```python
from build123d import *

# Parameters (mm, degrees)
SKETCH1_R           = 12.5
BOSS_EXTRUDE1_DEPTH = 10
M10_TAPPED_HOLE1_D  = 8.5
CHAMFER1_SIZE       = 2


with BuildPart() as part:
    # Sketch1 → Boss-Extrude1 (new, symmetric)
    with BuildSketch(Plane.XY):
        Circle(SKETCH1_R)
    extrude(amount=BOSS_EXTRUDE1_DEPTH, both=True)

    # M10 Tapped Hole1 (through all)
    with Locations(Plane.XY.offset(10)):
        with Locations((0, 0)):
            Hole(M10_TAPPED_HOLE1_D / 2)

    # Sketch5 → Revolve1 (revolve)
    with BuildSketch(Plane(origin=(0, 0, 0), x_dir=(1, 0, 0), z_dir=(0, 1, 0))):
        Polygon((-12.5, 0), (-92.29474156, 60.272707085), (-88.678379135, 65.060391578), (-8.883637575, 4.787684494), align=None)
    revolve(axis=Axis((-12.5, 0, 0), (-0.7979474156035873, 0, -0.6027270708467937)))

    # Chamfer1
    chamfer1_edges = [part.edges().sort_by_distance(p)[0] for p in [
        (-95.911103985, 0, -55.485022591),
    ]]
    chamfer(chamfer1_edges, length=CHAMFER1_SIZE)


solid = part.part
```
Source: CAD feature listing. Evaluate the final solid. Frame: model axes, mm. A direction names the side the tool comes from. Round coordinates to 2 decimals unless told otherwise and drop trailing zeros. Loops run counter-clockwise (first coordinate to the right, second up) from the corner with the lowest first, then second, coordinate; pieces in that order, holes last.
(1) Section query A-A (x = 0). Output: boundary loops of the cut face in (y, z), and give its area (3 significant figures).
From the geometry:
outline: (-12.5, -10) - (-4.25, -10) - (-4.25, 10) - (-12.5, 10) - close; (4.25, -10) - (12.5, -10) - (12.5, 10) - (4.25, 10) - close
area: 330 mm2
(2) Section query C-C (y = -7.25). Output: boundary loops of the cut face in (x, z).
From the geometry:
outline: (-10.18, -10) - (10.18, -10) - (10.18, 10) - (-10.18, 10) - close
(3) Pull-direction query (X, two-part tool) for faces 3 (the cylindrical face through (-2.285, 3.584, -0.14)), 4 (the flat face through (0, -5, 10)), 5 (the conical face through (-94.68, -0.18, -56.91)); classes: +X half, -X half, draft (parallel to the pull), parting line (faces both ways), or undercut.
From the geometry:
face 3: undercut
face 4: draft
face 5: -X half
(4) Section query B-B (y = 0). Output: boundary loops of the cut face in (x, z).
From the geometry:
outline: (-94.71, -57.08) - (-89.88, -63.46) - (-87.08, -63.85) - (-12.5, -7.52) - (-12.5, -10) - (-4.25, -10) - (-4.25, 10) - (-12.5, 10) - (-12.5, 0) - (-16.12, 4.79) - (-94.32, -54.28) - close; (4.25, -10) - (12.5, -10) - (12.5, 10) - (4.25, 10) - close
(5) Contact query for flat-ended pins moving along their axis: pin 1 Ø4 at (x, y) = (-25.5, 0) entering from -Z; pin 2 Ø5 at (y, z) = (1.5, -48) entering from -X; pin 3 Ø2 at (y, z) = (3, -29) entering from +X. Output: stop coordinate, or through.
From the geometry:
pin 1: stops at z = -18.85
pin 2: stops at x = -89.11
pin 3: stops at x = -40.7
(6) Material intervals for probe 1 along Y at (x, z) = (0, 2); probe 2 along Y at (x, z) = (-67, -41); probe 3 along Z at (x, y) = (-6.5, 9), sorted ascending.
From the geometry:
probe 1: y = -12.5 to -4.25, 4.25 to 12.5
probe 2: y = -6 to 6
probe 3: z = -10 to 10
(7) Access query for faces 1 (the flat face through (0, -5, -10)), 2 (the flat face through (-92.26, -0.06, -60.32)). Directions: +Z, -Z, +X, -X, +Y, -Y. A direction counts if a zero-diameter tool reaches every point of the face in a straight line with its end or side. Return the directions, or none.
From the geometry:
face 1: -Z, +X, +Y, -Y
face 2: -Z, -X, +Y, -Y
